Here's how the part is built. I have some questions about the finished solid (model axes, mm). A direction names the side the tool comes from. Round coordinates to 2 decimals unless told otherwise and drop trailing zeros. Write each loop counter-clockwise with the first axis right and the second up, starting at its lowest first coordinate (ties: lowest second). Pieces come first, ordered by that corner, then holes. Notation, with made-up numbers: (52, -23) -> (71, -23) arc R23 cw to (71, 14) -> close; hole circle Ø2 at (30.25, -34.5). An arc over 180 degrees is marked (long way). Answer in a Markdown table with one row per item. Add a question column.
from build123d import *

# Parameters (mm, degrees)
BOSS_EXTRUDE1_DEPTH                  = 8
F_16_0_16_DIAMETER_HOLE1_D           = 16
F_16_0_16_DIAMETER_HOLE2_D           = 16
F_16_0_16_DIAMETER_HOLE2_CSINK_D     = 19.6
F_16_0_16_DIAMETER_HOLE2_CSINK_ANGLE = 90
F_4_5_4_5_DIAMETER_HOLE1_D           = 4.5
CHAMFER1_SIZE                        = 1.5


with BuildPart() as part:
    # Sketch1 → Boss-Extrude1 (new body)
    with BuildSketch(Plane(origin=(8, 0, 0), x_dir=(0, 0, -1), z_dir=(1, 0, 0))):
        with BuildLine():
            Line((31, -19), (31, 19))
            ThreePointArc((31, 19), (0, 50), (-31, 19))
            Line((-31, 19), (-31, -19))
            ThreePointArc((-31, -19), (0, -50), (31, -19))
        make_face()
    extrude(amount=-BOSS_EXTRUDE1_DEPTH)

    # Sketch2 → Revolve1 (revolve)
    with BuildSketch(Plane.XY):
        Polygon((-27, 29), (-27, 19), (0, 19), (0, 30.786116689), (-15, 30), (-15, 29), align=None)
    revolve(axis=Axis((-27, 19, 0), (1, 0, 0)))

    # Ø16.0 (16) Diameter Hole1 (through all)
    with Locations(Plane.ZY):
        with Locations((0, -19)):
            Hole(F_16_0_16_DIAMETER_HOLE1_D / 2)

    # Ø16.0 (16) Diameter Hole2 (through all)
    with Locations(Plane.ZY.offset(27)):
        with Locations((0, 19)):
            CounterSinkHole(F_16_0_16_DIAMETER_HOLE2_D / 2, F_16_0_16_DIAMETER_HOLE2_CSINK_D / 2, counter_sink_angle=F_16_0_16_DIAMETER_HOLE2_CSINK_ANGLE)

    # Ø4.5 (4.5) Diameter Hole1 (through all)
    with Locations(Plane.ZY):
        with Locations((0, 46), (27, 19), (-27, 19), (27, -19), (-27, -19), (0, -46)):
            Hole(F_4_5_4_5_DIAMETER_HOLE1_D / 2)

    # Chamfer1
    chamfer1_edges = [part.edges().sort_by_distance(p)[0] for p in [
        (0, -46, 2.25),
        (0, -19, -24.75),
        (0, -19, 29.25),
        (0, 19, -24.75),
        (0, 19, 29.25),
        (0, 46, 2.25),
    ]]
    chamfer(chamfer1_edges, length=CHAMFER1_SIZE)


solid = part.part
Item 1: For P1, Ø18.5, axis at y = 19, z = 0, coming from the +X side; P2, Ø8, axis at x = 4, y = -30, coming from the -Z side; P3, Ø7, axis at y = 19, z = -27, coming from the -X side; P4, Ø4, axis at x = -16, z = -5, coming from the +Y side, each with a flat end and sliding along its axis, tell me the tip position at first contact or that it passes through.
Item 2: I need wall thicknesses on line 1 along Y through (x, z) = (5.5, 0); line 2 along Y through (x, z) = (5.5, -27); line 3 along X through (y, z) = (43.5, -6). Which ranges of each line are inside material? Lowest first, please. Write a range as from..to.
Item 3: If we section it at D-D on z = -27: Please give me the cut outline in (x, y), then the cut area to 3 significant figures.
Item 4: On a 3-axis mill with a long thin cutter (end or side, diameter ignored), from which of +Z, -Z, +X, -X, +Y, -Y can I reach the whole of each face in a straight line? I mean faces 1 (the cylindrical face through (4.795, 17.004, 25.962)), 2 (the flat face through (-15, 21, -10)). Say none if no direction works.
Item 5: If we section it at C-C on y = -46: Please give me the cut outline in (x, z).
Item 6: If we section it at A-A on z = 0: Give the number of separate pieces and of enclosed holes in the cut face, then the cut area to 3 significant figures.
Results list:
| question | item | result |
|---|---|---|
| 1 | P1 | x = 8 |
| 1 | P2 | z = -30.2 |
| 1 | P3 | x = 0.25 |
| 1 | P4 | y = 29.5 |
| 2 | line 1 | -50..-48.25, -43.75..-27, -11..11, 27..43.75, 48.25..50 |
| 2 | line 2 | -34.23..-21.25, -16.75..16.75, 21.25..34.23 |
| 2 | line 3 | 0..8 |
| 3 | outline | (0, -34.23) -> (8, -34.23) -> (8, -21.25) -> (1.5, -21.25) -> (0, -22.75) -> close; (0, -15.25) -> (1.5, -16.75) -> (8, -16.75) -> (8, 16.75) -> (1.5, 16.75) -> (0, 15.25) -> close; (0, 22.75) -> (1.5, 21.25) -> (8, 21.25) -> (8, 34.23) -> (0, 34.23) -> close |
| 3 | area | 471 mm² |
| 4 | face 1 | +X, -X |
| 4 | face 2 | -X |
| 5 | outline | (0, -15.23) -> (8, -15.23) -> (8, -2.25) -> (1.5, -2.25) -> (0, -3.75) -> close; (0, 3.75) -> (1.5, 2.25) -> (8, 2.25) -> (8, 15.23) -> (0, 15.23) -> close |
| 6 | separate pieces | 5 |
| 6 | enclosed holes | 0 |
| 6 | area | 614 mm² |
